```python
from build123d import *

# Parameters (mm, degrees)
SMALL_END_FLAT_DEPTH    = 10
BIG_END_FLAT_SKETCH_W   = 86.980428418
BIG_END_FLAT_SKETCH_H   = 55.493296348
BIG_END_FLAT_DEPTH      = 10
KEYED_BORE_20_DEPTH     = 40
SMALL_END_HOLE_SKETCH_R = 9
SMALL_END_HOLE_DEPTH    = 40
FILLET_R20_R            = 20
FILLET_R10_R            = 10
CROSS_HOLE_SKETCH_R     = 4
CROSS_HOLE_8_DEPTH      = 20


with BuildPart() as part:
    # Rod Profile Sketch → Rod Body Revolve (revolve)
    with BuildSketch(Plane.XY):
        with BuildLine():
            Line((-2.087121525, 10), (161.252272915, 10))
            ThreePointArc((161.252272915, 10), (180.257786585, 16.1664987), (192, 0))
            Line((192, 0), (-50, 0))
            ThreePointArc((-50, 0), (-30.107741092, 24.472657823), (-2.087121525, 10))
        make_face()
    revolve(axis=Axis((0, 0, 0), (1, 0, 0)))

    # Small End Flat Sketch → Small End Flat (cut)
    with BuildSketch(Plane(origin=(0, 7.5, 0), x_dir=(1, 0, 0), z_dir=(0, 1, 0))):
        Polygon((137.002179541, 20.26941877), (137.002179541, -16.521174788), (192.002179541, -16.521174788), (192.002179541, 18.008544306), align=None)
    small_end_flat = extrude(amount=SMALL_END_FLAT_DEPTH, mode=Mode.SUBTRACT)

    # Small End Flat Mirror: Small End Flat across plane
    add(small_end_flat.mirror(Plane.ZX), mode=Mode.SUBTRACT)

    # Big End Flat Sketch → Big End Flat (cut)
    with BuildSketch(Plane(origin=(0, 17.5, 0), x_dir=(1, 0, 0), z_dir=(0, 1, 0))):
        with Locations((-25, 0)):
            Rectangle(BIG_END_FLAT_SKETCH_W, BIG_END_FLAT_SKETCH_H)
    big_end_flat = extrude(amount=BIG_END_FLAT_DEPTH, mode=Mode.SUBTRACT)

    # Big End Flat Mirror: Big End Flat across plane
    add(big_end_flat.mirror(Plane.ZX), mode=Mode.SUBTRACT)

    # Keyed Bore Sketch → Keyed Bore Ø20 (cut)
    with BuildSketch(Plane(origin=(0, 17.5, 0), x_dir=(1, 0, 0), z_dir=(0, 1, 0))):
        with BuildLine():
            Line((-15.202041029, 2), (-12, 2))
            Line((-12, 2), (-12, -2))
            Line((-12, -2), (-15.202041029, -2))
            ThreePointArc((-15.202041029, -2), (-35, 0), (-15.202041029, 2))
        make_face()
    extrude(amount=-KEYED_BORE_20_DEPTH, mode=Mode.SUBTRACT)

    # Small End Hole Sketch → Small End Hole (cut)
    with BuildSketch(Plane(origin=(0, 7.5, 0), x_dir=(1, 0, 0), z_dir=(0, 1, 0))):
        with Locations(Location((175, 0, 0), (0, 0, 270))):
            Circle(SMALL_END_HOLE_SKETCH_R)
    extrude(amount=-SMALL_END_HOLE_DEPTH, mode=Mode.SUBTRACT)

    # Fillet R20
    fillet_r20_edges = [part.edges().sort_by_distance(p)[0] for p in [
        (-2.087121525, -10, 0),
    ]]
    fillet(fillet_r20_edges, radius=FILLET_R20_R)

    # Fillet R10
    fillet_r10_edges = [part.edges().sort_by_distance(p)[0] for p in [
        (161.252272915, 0, -10),
        (161.252272915, 0, 10),
    ]]
    fillet(fillet_r10_edges, radius=FILLET_R10_R)

    # Cross Hole Sketch → Cross Hole Ø8 (cut)
    with BuildSketch(Plane(origin=(-50, 0, 0), x_dir=(0, 0, -1), z_dir=(1, 0, 0))):
        with Locations(Location((0, 0, 0), (0, 0, 180))):
            Circle(CROSS_HOLE_SKETCH_R)
    extrude(amount=CROSS_HOLE_8_DEPTH, mode=Mode.SUBTRACT)


solid = part.part
```
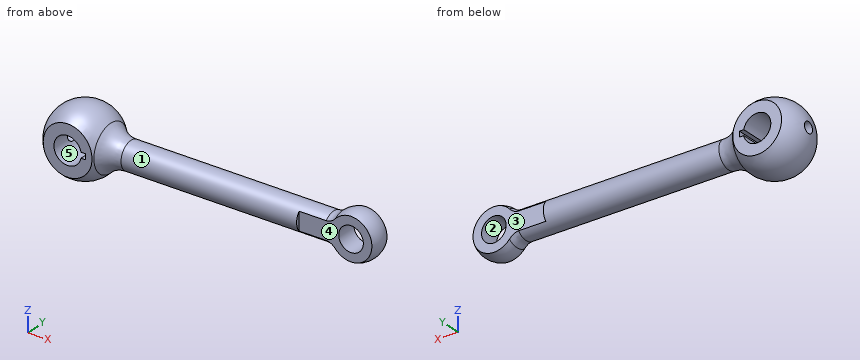
Part model, mm, in its own coordinate system. Face numbers are marked on the shaded views. A direction names the side the tool comes from. Round coordinates to 2 decimals unless told otherwise and drop trailing zeros. Loops run counter-clockwise (first coordinate to the right, second up) from the corner with the lowest first, then second, coordinate; pieces in that order, holes last.
Item 1: Mould opens along Z. For the marked faces 1, 2 and 3 say: +Z half, -Z half, draft (parallel to the pull), parting line (faces both ways), or undercut.
Item 2: Cut at B-B, the plane x = -25. Give the cut face in (y, z).
Item 3: Cut at A-A, the plane x = 175. Give the cut face in (y, z), then the cut area to 3 significant figures.
Item 4: 3-axis set-ups, long thin cutter, end or side, ignore diameter. For the marked faces 4 and 5: which of +Z, -Z, +X, -X, +Y, -Y reach the whole face in a straight line?
Item 5: Drill centre lines: line 1 (X direction, y = 0, z = 0); line 2 (X direction, y = 5.5, z = 0); line 3 (Z direction, x = -25, y = -7). Where is each one in solid material? Low to high.
Item 6: Drop flat-ended pins along their axis: P1, Ø1, axis at x = 111, y = -6, coming from the -Z side; P2, Ø10, axis at x = 161, y = -2.5, coming from the +Z side; P3, Ø3, axis at x = 47, z = -1.5, coming from the -Y side. Give the stop position or say it passes through.
A:
1. face 1: parting line
1. face 2: undercut
1. face 3: draft
2. outline: (-17.5, -17.85) arc R25 ccw to (17.5, -17.85) - (17.5, -10) - (-17.5, -10) - close; (-17.5, 10) - (17.5, 10) - (17.5, 17.85) arc R25 ccw to (-17.5, 17.85) - close
3. outline: (-7.5, -15.26) arc R17 ccw to (7.5, -15.26) - (7.5, -9) - (-7.5, -9) - close; (-7.5, 9) - (7.5, 9) - (7.5, 15.26) arc R17 ccw to (-7.5, 15.26) - close
3. area: 223 mm2
4. face 4: +Z, -Z, +X, -Y
4. face 5: +Y, -Y
5. line 1: x = -12 to 166, 184 to 192
5. line 2: x = -49.39 to -35, -12 to 166, 184 to 191.09
5. line 3: z = -24 to -10, 10 to 24
6. P1: stops at z = -8.35
6. P2: stops at z = 14.28
6. P3: stops at y = -10
